The figure shows three views and two pictorial views of one solid part (mm, origin at its lowest corner). Answer the questions. Give positions to 0.01 mm unless a question says otherwise; leave off trailing zeros. Order: outer loops, then holes, each group sorted by start corner. A loop starts at its lowest first (then second) coordinate and runs counter-clockwise, first axis right, second up. Notation, with made-up numbers: M 43,29 L 58,29 A27 ccw 58,57 Z; hole C 83.25,22 d1. An arc over 180 degrees is marked long. One line per item, written item: value. Start each with the question number.
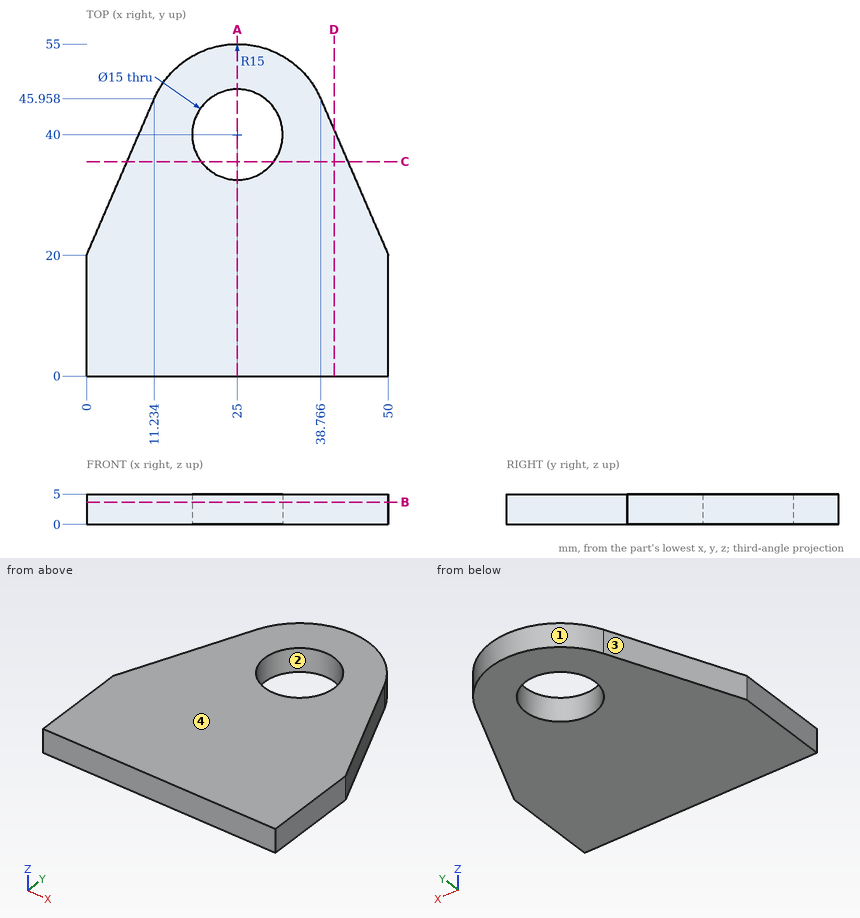
Q1. Find section D-D, the plane x = 41. Give the vertices of the cut face in (y, z), then the cut area to 3 significant figures.
Q2. Find section C-C, the plane y = 35.5. Give the vertices of the cut face in (x, z), then the cut area to 3 significant figures.
Q3. Determine the mould class of the marked faces 1, 2, 3 and 4 for opening direction X: released by +X, released by -X, zero draft, split by the parting line, or undercut.
Q4. Consider probe 1 along Y at (x, z) = (25, 2.35); probe 2 along Y at (x, z) = (23, 4.2); probe 3 along Y at (x, z) = (46, 1.65) (1 decimal). Determine where each line is inside the solid, lowest interval first.
Q5. Find section B-B, the plane z = 3.65. Give the vertices of the cut face in (x, y), then the cut area to 3 significant figures.
Q6. This flat-tipped pin is pushed along its axis until it touches: pin 1 (2 mm diameter, centred on y = 45, z = 2, fed in from -X). Where does it stop, or does it pass through?
Q7. Find section A-A, the plane x = 25. Give the vertices of the cut face in (y, z), then the cut area to 3 significant figures.
Evaluation:
1. outline: M 0,0 L 40.8,0 L 40.8,5 L 0,5 Z
1. area: 204 mm2
2. outline: M 6.71,0 L 19,0 L 19,5 L 6.71,5 Z; M 31,0 L 43.29,0 L 43.29,5 L 31,5 Z
2. area: 123 mm2
3. face 1: split by the parting line
3. face 2: undercut
3. face 3: released by -X
3. face 4: zero draft
4. probe 1: 0 to 32.5, 47.5 to 55
4. probe 2: 0 to 32.77, 47.23 to 54.87
4. probe 3: 0 to 29.2
5. outline: M 0,0 L 50,0 L 50,20 L 38.77,45.96 A15 ccw 11.23,45.96 L 0,20 Z; hole C 25,40 d15
5. area: 2,010 mm2
6. pin 1: x = 10.39
7. outline: M 0,0 L 32.5,0 L 32.5,5 L 0,5 Z; M 47.5,0 L 55,0 L 55,5 L 47.5,5 Z
7. area: 200 mm2
